Read the model definition and answer for the solid it produces. Units are mm, in the model's axes. Face numbers are marked on the shaded views. A direction names the side the tool comes from. Give positions to 0.01 mm unless a question says otherwise; leave off trailing zeros. Order: outer loops, then holes, each group sorted by start corner. A loop starts at its lowest first (then second) coordinate and runs counter-clockwise, first axis right, second up. Notation, with made-up numbers: (9.25, 6.5) - (62.25, 6.5) arc R12 ccw to (62.25, 12.5) - close; hole circle Ø3 at (44, 2). An arc over 180 degrees is marked (long way). Use a Markdown table: item, result. Add a question column.
1. Flat-ended cylindrical pins translate along their axes: P1, Ø1.5, axis at x = 11, z = -15, coming from the -Y side; P2, Ø10, axis at x = -0.5, y = 12, coming from the +Z side; P3, Ø1, axis at x = 8.5, z = -5, coming from the +Y side; P4, Ø10, axis at x = 14, z = -8, coming from the +Y side. Find the tip coordinate at first contact, or state that the pin passes through.
2. Which of the six approach directions +Z, -Z, +X, -X, +Y, -Y give full straight-line access (tool end or side, diameter ignored) to the marked faces 1 and 2?
3. A cutting plane is placed at A-A on z = -21.25. Determine the outline of the cut face in (x, y) (1 decimal), and give its area (3 significant figures).
4. Consider L1, parallel to Y at x = 0, z = -17.75 (3 decimals); L2, parallel to Y at x = -5, z = -10.5; L3, parallel to Z at x = -15, y = -15.5. Determine where each line is inside the solid, lowest interval first.
5. For a pull along X with two mould halves and no side action, classify the marked faces 3, 4 and 5 as released by +X, released by -X, zero draft, split by the parting line, or undercut.
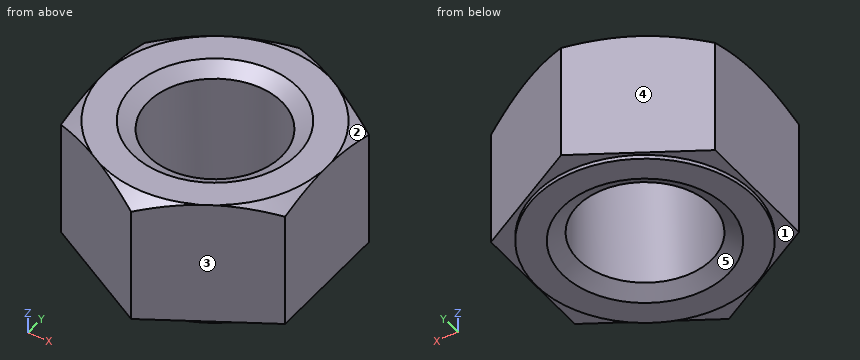
```python
from build123d import *

# Parameters (mm, degrees)
SKETCH_3_R          = 13.105625
EXTRUDE_1_DEPTH     = 25.6
SKETCH_5_R          = 38.1375
SKETCH_5_R_2        = 22.018695891
CUT_EXTRUDE_1_DEPTH = 5.12
CUT_EXTRUDE_1_DRAFT = -60
SKETCH_6_W          = 0.8
SKETCH_6_H          = 4.025


with BuildPart() as part:
    # 草图3 → 凸台-拉伸1 (new body)
    with BuildSketch(Plane.XY):
        Polygon((0, 25.425), (-22.018695891, 12.7125), (-22.018695891, -12.7125), (0, -25.425), (22.018695891, -12.7125), (22.018695891, 12.7125), align=None)
        Circle(SKETCH_3_R, mode=Mode.SUBTRACT)
    extrude(amount=-EXTRUDE_1_DEPTH)

    # 草图4 → 切除-旋转1 (revolve, cut)
    with BuildSketch(Plane(origin=(0, 0, 0), x_dir=(0, 0, -1), z_dir=(1, 0, 0)), mode=Mode.PRIVATE) as cut_revolve_1_sk:
        Polygon((0, 16.2), (1.786538239, 13.105625), (1.786538239, 0), (0, 0), align=None)
        Polygon((25.6, 0), (25.6, 16.2), (23.813461761, 13.105625), (23.813461761, 0), align=None)
    revolve(cut_revolve_1_sk.sketch.rotate(Axis((0, 0, 0), (0, 0, -1)), 90), axis=Axis((0, 0, 0), (0, 0, -1)), mode=Mode.SUBTRACT)


with BuildPart() as cut_extrude_1_tool:
    # 草图5 → 切除-拉伸1 (with draft: the straight prism first)
    with BuildSketch(Plane.XY):
        Circle(SKETCH_5_R)
        Circle(SKETCH_5_R_2, mode=Mode.SUBTRACT)
    extrude(amount=-CUT_EXTRUDE_1_DEPTH)
    # 切除-拉伸1: the draft: its side faces are tilted about the plane it starts from
    cut_extrude_1_sides = [cut_extrude_1_tool.faces().sort_by_distance(p)[0] for p in [
        (-38.1375, 0, -2.56),
        (-22.018695891, 0, -2.56),
    ]]
    draft(cut_extrude_1_sides, Plane.XY, CUT_EXTRUDE_1_DRAFT)


with BuildPart() as part_1:
    add(part.part)

    # 切除-拉伸1: cut by cut_extrude_1_tool
    add(cut_extrude_1_tool.part, mode=Mode.SUBTRACT)

    # 草图6 → 切除-旋转2 (revolve, cut)
    with BuildSketch(Plane(origin=(0, 0, 0), x_dir=(0, 0, -1), z_dir=(1, 0, 0)), mode=Mode.PRIVATE) as cut_revolve_2_sk:
        with Locations((25.2, 23.4125)):
            Rectangle(SKETCH_6_W, SKETCH_6_H)
    revolve(cut_revolve_2_sk.sketch.rotate(Axis((0, 0, 0), (0, 0, -1)), 90), axis=Axis((0, 0, 0), (0, 0, -1)), mode=Mode.SUBTRACT)


solid = part_1.part
```
Output values:
| question | item | result |
|---|---|---|
| 1 | P1 | y = -19.51 |
| 1 | P2 | z = 0 |
| 1 | P3 | y = 20.81 |
| 1 | P4 | y = 20.23 |
| 2 | face 1 | -Z |
| 2 | face 2 | +Z, +X, +Y |
| 3 | outline | (-22, -12.7) - (0, -25.4) - (22, -12.7) - (22, 12.7) - (0, 25.4) - (-22, 12.7) - close; hole circle Ø26.2 at (0, 0) |
| 3 | area | 1,140 mm² |
| 4 | L1 | -25.425 to -13.106, 13.106 to 25.425 |
| 4 | L2 | -22.54 to -12.11, 12.11 to 22.54 |
| 4 | L3 | -24.8 to 0 |
| 5 | face 3 | released by +X |
| 5 | face 4 | released by -X |
| 5 | face 5 | undercut |
